```python
from build123d import *

# Parameters (mm, degrees)
MAIN_BOSS_SKETCH_32_R    = 16
MAIN_BOSS_32_DEPTH       = 17.5
MAIN_BOSS_BORE_SKETCH_R  = 8.5
MAIN_BOSS_BORE_DEPTH     = 57
LOWER_ARM_PLATE_DEPTH    = 4
UPPER_BOSS_SKETCH_R      = 16
UPPER_BOSS_DEPTH         = 33
UPPER_BOSS_BORE_SKETCH_R = 8.5
UPPER_BOSS_BORE_DEPTH    = 38
UPPER_ARM_PLATE_DEPTH    = 8
PLATE_CUT_SET_A_DEPTH    = 38
PLATE_CUT_SET_B_DEPTH    = 38
RIB_DEPTH                = 3.5
RIB_FILLET_R5_R          = 5
ARM_JUNCTION_FILLET_R3_R = 3
GUSSET_SKETCH_W          = 58
GUSSET_SKETCH_H          = 10
GUSSET_DEPTH             = 55
GUSSET_TRIM_SKETCH_R     = 9
GUSSET_TRIM_CUT_DEPTH    = 55


with BuildPart() as part:
    # Main Boss Sketch Ø32 → Main Boss Ø32 (new, symmetric)
    with BuildSketch(Plane(origin=(0, 0, 0), x_dir=(1, 0, 0), z_dir=(0, 1, 0))):
        with Locations(Location((0, 0, 0), (0, 0, 270))):
            Circle(MAIN_BOSS_SKETCH_32_R)
    extrude(amount=MAIN_BOSS_32_DEPTH, both=True)

    # Main Boss Bore Sketch → Main Boss Bore (cut)
    with BuildSketch(Plane(origin=(0, 17.5, 0), x_dir=(1, 0, 0), z_dir=(0, 1, 0))):
        with Locations(Location((0, 0, 0), (0, 0, 270))):
            Circle(MAIN_BOSS_BORE_SKETCH_R)
    extrude(amount=-MAIN_BOSS_BORE_DEPTH, mode=Mode.SUBTRACT)

    # Lower Arm Sketch → Lower Arm Plate (add, symmetric)
    with BuildSketch(Plane(origin=(0, 0, 0), x_dir=(1, 0, 0), z_dir=(0, 1, 0))):
        with BuildLine():
            Line((0, 81), (29, 81))
            Line((29, 81), (16, 0))
            ThreePointArc((16, 0), (0, 16), (-16, 0))
            Line((-16, 0), (-29, 81))
            Line((-29, 81), (0, 81))
        make_face()
    extrude(amount=LOWER_ARM_PLATE_DEPTH, both=True)



with BuildPart() as body_2:
    # Upper Boss Sketch → Upper Boss (new body)
    with BuildSketch(Plane.XY.offset(-48)):
        with Locations((0, 52.5)):
            Circle(UPPER_BOSS_SKETCH_R)
    extrude(amount=-UPPER_BOSS_DEPTH)

    # Upper Boss Bore Sketch → Upper Boss Bore (cut)
    with BuildSketch(Plane.XY.offset(-48)):
        with Locations((0, 52.5)):
            Circle(UPPER_BOSS_BORE_SKETCH_R)
    extrude(amount=-UPPER_BOSS_BORE_DEPTH, mode=Mode.SUBTRACT)


with BuildPart() as part_1:
    add(part.part)

    add(body_2.part)  # Upper Arm Plate merges body 2
    # Upper Arm Sketch → Upper Arm Plate (add)
    with BuildSketch(Plane.XY.offset(-65)):
        with BuildLine():
            Line((-26.431737368, 4), (29, 4))
            Line((29, 4), (16, 52.5))
            ThreePointArc((16, 52.5), (0, 36.5), (-16, 52.5))
            Line((-16, 52.5), (-29, 4))
            Line((-29, 4), (-26.431737368, 4))
        make_face()
    extrude(amount=-UPPER_ARM_PLATE_DEPTH)

    # Plate Cut Set A Sketch → Plate Cut Set A (cut)
    with BuildSketch(Plane.XZ.offset(4)):
        Polygon((27.716049383, -73), (26.432098765, -65), (29, -65), (29, -73), align=None)
    extrude(amount=-PLATE_CUT_SET_A_DEPTH, mode=Mode.SUBTRACT)

    # Plate Cut Set B Sketch → Plate Cut Set B (cut)
    with BuildSketch(Plane.XZ.offset(4)):
        Polygon((-26.432098765, -65), (-29, -65), (-29, -73), (-27.716049383, -73), align=None)
    extrude(amount=-PLATE_CUT_SET_B_DEPTH, mode=Mode.SUBTRACT)

    # Rib Sketch → Rib (add, symmetric)
    with BuildSketch(Plane(origin=(0, 0, 0), x_dir=(0, 0, -1), z_dir=(1, 0, 0))):
        Polygon((48, 17.5), (11.269108444, 17.5), (11.269108444, 4), (65, 4), (65, 40.002332079), (48, 40.002332079), align=None)
    extrude(amount=RIB_DEPTH, both=True)

    # Rib Fillet R5
    rib_fillet_r5_edges = [part_1.edges().sort_by_distance(p)[0] for p in [
        (0, 17.5, -48),
    ]]
    fillet(rib_fillet_r5_edges, radius=RIB_FILLET_R5_R)

    # Arm Junction Fillet R3
    arm_junction_fillet_r3_edges = [part_1.edges().sort_by_distance(p)[0] for p in [
        (14.966049383, 4, -65),
    ]]
    fillet(arm_junction_fillet_r3_edges, radius=ARM_JUNCTION_FILLET_R3_R)

    # Gusset Sketch → Gusset (add)
    with BuildSketch(Plane.XZ.offset(4)):
        with Locations((0, -76)):
            Rectangle(GUSSET_SKETCH_W, GUSSET_SKETCH_H)
    extrude(amount=GUSSET_DEPTH)

    # Gusset Trim Sketch → Gusset Trim Cut (cut)
    with BuildSketch(Plane.XY.offset(-71)):
        with Locations((19, -44)):
            Circle(GUSSET_TRIM_SKETCH_R)
        with Locations((19, -19)):
            Circle(GUSSET_TRIM_SKETCH_R)
        with Locations((-19, -44)):
            Circle(GUSSET_TRIM_SKETCH_R)
        with Locations((-19, -19)):
            Circle(GUSSET_TRIM_SKETCH_R)
    extrude(amount=-GUSSET_TRIM_CUT_DEPTH, mode=Mode.SUBTRACT)


solid = part_1.part
```
Can you work these out from the model? Positions are in its coordinate system, mm. A direction names the side the tool comes from. Give positions to 0.01 mm unless a question says otherwise; leave off trailing zeros. Order: outer loops, then holes, each group sorted by start corner. A loop starts at its lowest first (then second) coordinate and runs counter-clockwise, first axis right, second up. Notation, with made-up numbers: (10, -4) - (14, -4) arc R24 ccw to (14, 33) - close; hole circle Ø8 at (80.5, 69). An arc over 180 degrees is marked (long way). Use a Markdown table: item, result. Add a question column.
Q1. If we mould it in two halves opening along X, with no side actions, what happens to faces 4 (the flat face through (29, -31, -76)), 5 (the flat face through (-15, 23, -65)), 6 (the flat face through (-3.5, 17, -45)), 7 (the cylindrical face through (8.428, 0.245, -1.107))? For each: released by +X, released by -X, zero draft, split by the parting line, or undercut.
Q2. I'm going to push flat-ended pins straight in: pin 1 (3 mm diameter, centred on x = 10.5, z = -40, fed in from -Y); pin 2 (6 mm diameter, centred on x = -14.5, z = -58.5, fed in from +Y); pin 3 (7 mm diameter, centred on x = -11.5, z = -48.5, fed in from +Y); pin 4 (16 mm diameter, centred on x = -19, y = -44, fed in from -Z). Where does each tip first touch, or does it pass through?
Q3. On a 3-axis mill with a long thin cutter (end or side, diameter ignored), from which of +Z, -Z, +X, -X, +Y, -Y can I reach the whole of each face in a straight line? I mean faces 1 (the flat face through (0, 4, -77)), 2 (the flat face through (0, 17.5, -14)), 3 (the flat face through (0, -31, -71)). Say none if no direction works.
Q4. Please list where these lines run through material, in increasing order: line 1 along Y through (x, z) = (19, -77.75); line 2 along X through (y, z) = (8.5, 0); line 3 along Y through (x, z) = (6.5, -51.5).
Q5. If we section it at B-B on z = 1.5: Write out the boundary of the cut face in (x, y), plus the area to 3 significant figures.
Q6. If we section it at C-C on x = 0: Write out the boundary of the cut face in (y, z), plus the area to 3 significant figures.
Q7. If we section it at D-D on y = -44: Write out the boundary of the cut face in (x, z).
Q8. If we section it at A-A on y = -7.5: Write out the boundary of the cut face in (x, z).
Answers follow:
| question | item | result |
|---|---|---|
| 1 | face 4 | released by +X |
| 1 | face 5 | zero draft |
| 1 | face 6 | released by -X |
| 1 | face 7 | undercut |
| 2 | pin 1 | stops at y = -4 |
| 2 | pin 2 | stops at y = 63.62 |
| 2 | pin 3 | stops at y = 66.36 |
| 2 | pin 4 | passes through |
| 3 | face 1 | -Z, +X, -X |
| 3 | face 2 | +Z, +X, -X, +Y |
| 3 | face 3 | +X, -X, -Y |
| 4 | line 1 | y = -59 to -53, -35 to -28, -10 to 4 |
| 4 | line 2 | x = -16 to -8.5, 8.5 to 16 |
| 4 | line 3 | y = -4 to 4, 37.88 to 47.02, 57.98 to 67.12 |
| 5 | outline | (-15.93, -17.5) - (-8.37, -17.5) - (-8.37, 17.5) - (-15.93, 17.5) - close; (8.37, -17.5) - (15.93, -17.5) - (15.93, 17.5) - (8.37, 17.5) - close |
| 5 | area | 529 mm^2 |
| 6 | outline | (-59, -81) - (4, -81) - (4, -73) - (36.5, -73) - (36.5, -81) - (44, -81) - (44, -48) - (22.5, -48) arc R5 cw to (17.5, -43) - (17.5, -8.5) - (-17.5, -8.5) - (-17.5, -16) - (-4, -16) - (-4, -71) - (-59, -71) - close; (-17.5, 8.5) - (17.5, 8.5) - (17.5, 16) - (-17.5, 16) - close; (61, -81) - (68.5, -81) - (68.5, -48) - (61, -48) - close |
| 6 | area | 3,340 mm^2 |
| 7 | outline | (-29, -81) - (-28, -81) - (-28, -71) - (-29, -71) - close; (-10, -81) - (10, -81) - (10, -71) - (-10, -71) - close; (28, -81) - (29, -81) - (29, -71) - (28, -71) - close |
| 8 | outline | (-29, -81) - (29, -81) - (29, -71) - (-29, -71) - close; circle Ø32 at (0, 0); hole circle Ø17 at (0, 0) |
